from build123d import *

# Parameters (mm, degrees)
SKETCH_1_R          = 28
EXTRUDE_1_DEPTH     = 40
EXTRUDE_2_DEPTH     = 16
SKETCH_3_R          = 20
CUT_EXTRUDE_1_DEPTH = 71.604532432
SKETCH_4_R          = 6
CUT_EXTRUDE_2_DEPTH = 63.93647591


with BuildPart() as part:
    # 草图1 → 凸台-拉伸1 (new body)
    with BuildSketch(Plane(origin=(0, 0, 0), x_dir=(1, 0, 0), z_dir=(0, 1, 0))):
        with Locations(Location((0, 0, 0), (0, 0, 270))):
            Circle(SKETCH_1_R)
    extrude(amount=EXTRUDE_1_DEPTH)

    # 草图2 → 凸台-拉伸2 (add)
    with BuildSketch(Plane.XZ):
        Polygon((-51, -12.5), (-51, 12.5), (-8.862653898, 26.560372096), (-8.862653898, -26.560372096), align=None)
    extrude_2 = extrude(amount=-EXTRUDE_2_DEPTH)

    # 镜向1: 凸台-拉伸2 across plane
    add(extrude_2.mirror(Plane(origin=(0, 0, 0), x_dir=(0, 0, 1), z_dir=(1, 0, 0))))

    # 草图3 → 切除-拉伸1 (cut, through all)
    with BuildSketch(Plane(origin=(0, 40, 0), x_dir=(1, 0, 0), z_dir=(0, 1, 0))):
        with Locations(Location((0, 0, 0), (0, 0, 270))):
            Circle(SKETCH_3_R)
    extrude(amount=-CUT_EXTRUDE_1_DEPTH, mode=Mode.SUBTRACT)

    # 草图4 → 切除-拉伸2 (cut, through all)
    with BuildSketch(Plane(origin=(0, 16, 0), x_dir=(1, 0, 0), z_dir=(0, 1, 0))):
        with Locations(Location((-40, 0, 0), (0, 0, 270))):
            Circle(SKETCH_4_R)
        with Locations(Location((40, 0, 0), (0, 0, 270))):
            Circle(SKETCH_4_R)
    extrude(amount=-CUT_EXTRUDE_2_DEPTH, mode=Mode.SUBTRACT)


solid = part.part
Can you work these out from the model? Positions are in its coordinate system, mm. A direction names the side the tool comes from. Round coordinates to 2 decimals unless told otherwise and drop trailing zeros. Order: outer loops, then holes, each group sorted by start corner. A loop starts at its lowest first (then second) coordinate and runs counter-clockwise, first axis right, second up. Notation, with made-up numbers: (-12.75, -27.75) -> (-8.75, -27.75) arc R31 cw to (-8.75, 10.25) -> close; hole circle Ø7 at (-2.5, 71). An arc over 180 degrees is marked (long way). Write each question's results on one line, items separated by ' | '. Start each with the question number.
Item 1: If we section it at A-A, the plane x = 0: Write out the boundary of the cut face in (y, z).
Item 2: If we section it at C-C, the plane z = 5: Write out the boundary of the cut face in (x, y).
Item 3: If we section it at D-D, the plane z = 14.5: Write out the boundary of the cut face in (x, y), then the cut area to 3 significant figures.
Item 4: Thinking about a two-plate mould opening in X: for faces 3 (the flat face through (51, 8, 0)), 4 (the cylindrical face through (-45.857, 8.112, -1.301)), 5 (the flat face through (19, 40, -7)), which applies, +X half, -X half, draft (parallel to the pull), parting line (faces both ways), or undercut?
Item 5: Which directions (+Z, -Z, +X, -X, +Y, -Y) give clear straight access to the entire face, cutting with the end or side of a thin tool? Please do faces 1 (the cylindrical face through (27.76, 24.16, -3.65)), 2 (the flat face through (29.636, 7.888, -19.629)).
Item 6: Will these pins go through, and if not, where does the flat tip stop? pin 1 (19 mm diameter, centred on x = 40, z = 0, fed in from -Y); pin 2 (10 mm diameter, centred on y = 21.5, z = -3.5, fed in from -X); pin 3 (3 mm diameter, centred on x = 19, y = 24.5, fed in from +Z).
Item 7: If we section it at B-B, the plane y = 7: Write out the boundary of the cut face in (x, z), then the cut area to 3 significant figures.
Item 8: Please list where these lines run through material, in increasing order: L1, parallel to X at y = 7.25, z = 0; L2, parallel to X at y = 24, z = 0; L3, parallel to Z at x = 16, y = 27.5.
Results:
1) outline: (0, -28) -> (40, -28) -> (40, -20) -> (0, -20) -> close; (0, 20) -> (40, 20) -> (40, 28) -> (0, 28) -> close
2) outline: (-51, 0) -> (-43.32, 0) -> (-43.32, 16) -> (-51, 16) -> close; (-36.68, 0) -> (-19.36, 0) -> (-19.36, 40) -> (-27.55, 40) -> (-27.55, 16) -> (-36.68, 16) -> close; (19.36, 0) -> (36.68, 0) -> (36.68, 16) -> (27.55, 16) -> (27.55, 40) -> (19.36, 40) -> close; (43.32, 0) -> (51, 0) -> (51, 16) -> (43.32, 16) -> close
3) outline: (-45.01, 0) -> (-13.77, 0) -> (-13.77, 40) -> (-23.95, 40) -> (-23.95, 16) -> (-45.01, 16) -> close; (13.77, 0) -> (45.01, 0) -> (45.01, 16) -> (23.95, 16) -> (23.95, 40) -> (13.77, 40) -> close | area: 1,490 mm2
4) face 3: +X half | face 4: undercut | face 5: draft
5) face 1: +Y | face 2: -Z, +X, +Y, -Y
6) pin 1: stops at y = 0 | pin 2: stops at x = -28 | pin 3: stops at z = 21.86
7) outline: (-51, -12.5) -> (-8.86, -26.56) arc R28 ccw to (8.86, -26.56) -> (51, -12.5) -> (51, 12.5) -> (8.86, 26.56) arc R28 ccw to (-8.86, 26.56) -> (-51, 12.5) -> close; hole circle Ø12 at (-40, 0); hole circle Ø40 at (0, 0); hole circle Ø12 at (40, 0) | area: 2,780 mm2
8) L1: x = -51 to -46, -34 to -20, 20 to 34, 46 to 51 | L2: x = -28 to -20, 20 to 28 | L3: z = -22.98 to -12, 12 to 22.98
